Read the model definition and answer for the solid it produces. Units are mm, in the model's axes. A direction names the side the tool comes from. Round coordinates to 2 decimals unless told otherwise and drop trailing zeros. Loops run counter-clockwise (first coordinate to the right, second up) from the corner with the lowest first, then second, coordinate; pieces in that order, holes last. Notation, with made-up numbers: M 66,75 L 113,75 A34 ccw 113,114 Z; hole C 33,-29.5 d8. An arc over 180 degrees is marked long. Write each question's results on one line, items separated by ' | '.
```python
from build123d import *

# Parameters (mm, degrees)
SKETCH1_W                                         = 71.5
SKETCH1_H                                         = 30
SKETCH1_W_2                                       = 63.5
SKETCH1_H_2                                       = 22
BOSS_EXTRUDE1_DEPTH                               = 21
SKETCH2_W                                         = 71.5
SKETCH2_H                                         = 30
BOSS_EXTRUDE2_DEPTH                               = 3
SKETCH3_W                                         = 68.9
SKETCH3_H                                         = 27.4
SKETCH3_W_2                                       = 65.9
SKETCH3_H_2                                       = 24.4
CUT_EXTRUDE1_DEPTH                                = 1.5
SKETCH4_R                                         = 1.6
CUT_EXTRUDE2_DEPTH                                = 3
PILOT_HOLE_SIZE_PER_CROSS_FOR_HALF_CO_D           = 3.2
PILOT_HOLE_SIZE_PER_CROSS_FOR_HALF_CO_DEPTH       = 6.1
PILOT_HOLE_SIZE_PER_CROSS_FOR_HALF_CO_CSINK_D     = 6
PILOT_HOLE_SIZE_PER_CROSS_FOR_HALF_CO_CSINK_ANGLE = 90
PILOT_HOLE_SIZE_PER_CROSS_FOR_HALF_CO_TIP         = 0.96137699
FILLET1_R                                         = 1
FILLET2_R                                         = 1


with BuildPart() as part:
    # Sketch1 → Boss-Extrude1 (new body)
    with BuildSketch(Plane.XY):
        Rectangle(SKETCH1_W, SKETCH1_H)
        Rectangle(SKETCH1_W_2, SKETCH1_H_2, mode=Mode.SUBTRACT)
    extrude(amount=BOSS_EXTRUDE1_DEPTH)

    # Sketch2 → Boss-Extrude2 (add)
    with BuildSketch(Plane.XY.offset(21)):
        Polygon((42.25, 15), (42.25, -15), (42.25, -21.5), (-42.25, -21.5), (-42.25, -15), (-42.25, 15), (-42.25, 21.5), (42.25, 21.5), align=None)
        Rectangle(SKETCH2_W, SKETCH2_H, mode=Mode.SUBTRACT)
    extrude(amount=-BOSS_EXTRUDE2_DEPTH)

    # Sketch3 → Cut-Extrude1 (cut)
    with BuildSketch(Plane(origin=(0, 0, 0), x_dir=(-1, 0, 0), z_dir=(0, 0, -1))):
        Rectangle(SKETCH3_W, SKETCH3_H)
        Rectangle(SKETCH3_W_2, SKETCH3_H_2, mode=Mode.SUBTRACT)
    extrude(amount=-CUT_EXTRUDE1_DEPTH, mode=Mode.SUBTRACT)

    # Sketch4 → Cut-Extrude2 (cut)
    with BuildSketch(Plane(origin=(0, 0, 18), x_dir=(-1, 0, 0), z_dir=(0, 0, -1))):
        with Locations((-38.25, 16.5)):
            Circle(SKETCH4_R)
        with Locations((-38.25, -16.5)):
            Circle(SKETCH4_R)
        with Locations(Location((38.25, -16.5, 0), (0, 0, 180))):
            Circle(SKETCH4_R)
        with Locations(Location((38.25, 16.5, 0), (0, 0, 180))):
            Circle(SKETCH4_R)
        with Locations((0, -18)):
            Circle(SKETCH4_R)
        with Locations((0, 18)):
            Circle(SKETCH4_R)
    extrude(amount=-CUT_EXTRUDE2_DEPTH, mode=Mode.SUBTRACT)

    # Pilot hole size (% per cross) for half-countersunk wood screw, type 1
    with Locations(Plane.XY.offset(21)):
        with Locations((-38.25, 16.5), (-38.25, -16.5), (38.25, 16.5), (38.25, -16.5), (0, -18), (0, 18)):
            CounterSinkHole(PILOT_HOLE_SIZE_PER_CROSS_FOR_HALF_CO_D / 2, PILOT_HOLE_SIZE_PER_CROSS_FOR_HALF_CO_CSINK_D / 2, depth=PILOT_HOLE_SIZE_PER_CROSS_FOR_HALF_CO_DEPTH, counter_sink_angle=PILOT_HOLE_SIZE_PER_CROSS_FOR_HALF_CO_CSINK_ANGLE)
            with Locations((0, 0, -(PILOT_HOLE_SIZE_PER_CROSS_FOR_HALF_CO_DEPTH + PILOT_HOLE_SIZE_PER_CROSS_FOR_HALF_CO_TIP / 2))):  # 118° drill point
                Cone(0, PILOT_HOLE_SIZE_PER_CROSS_FOR_HALF_CO_D / 2, PILOT_HOLE_SIZE_PER_CROSS_FOR_HALF_CO_TIP, mode=Mode.SUBTRACT)

    # Fillet1
    fillet1_edges = [part.edges().sort_by_distance(p)[0] for p in [
        (-31.75, 11, 10.5),
        (-31.75, -11, 10.5),
        (31.75, -11, 10.5),
        (31.75, 11, 10.5),
        (34.45, 13.7, 0.75),
        (-34.45, 13.7, 0.75),
        (-34.45, -13.7, 0.75),
        (34.45, -13.7, 0.75),
        (32.95, -12.2, 0.75),
        (32.95, 12.2, 0.75),
        (-32.95, 12.2, 0.75),
        (-32.95, -12.2, 0.75),
    ]]
    fillet(fillet1_edges, radius=FILLET1_R)

    # Fillet2
    fillet2_edges = [part.edges().sort_by_distance(p)[0] for p in [
        (-35.75, -15, 9),
        (-35.75, 15, 9),
        (35.75, 15, 9),
        (35.75, -15, 9),
    ]]
    fillet(fillet2_edges, radius=FILLET2_R)


solid = part.part
```
1. Given P1, Ø1.6, axis at x = -2, z = 1, coming from the +Y side; P2, Ø3, axis at y = 11, z = 13.5, coming from the +X side; P3, Ø5, axis at x = -38.25, y = 16.5, coming from the +Z side, each flat-ended and moving along its own axis, determine where each tip first touches the part or whether it passes through.
Completed:
P1: stops at y = 15 | P2: stops at x = 35.75 | P3: stops at z = 20.5
2. Find the intervals of material crossed by L1, parallel to Y at x = -38.25, z = 19.2; L2, parallel to Y at x = 0, z = 19.15; L3, parallel to Y at x = 8.5, z = 2.5, in increasing order.
Completed:
L1: y = -21.5 to -18.1, -14.9 to 14.9, 18.1 to 21.5 | L2: y = -21.5 to -19.6, -16.4 to -11, 11 to 16.4, 19.6 to 21.5 | L3: y = -15 to -11, 11 to 15
3. Find section B-B, the plane x = 0. Count the separate pieces of the cut face and the enclosed holes in it, then the cut area to 3 significant figures.
Completed:
separate pieces: 4 | enclosed holes: 0 | area: 179 mm2
4. Find section C-C, the plane z = 12.5. Give the vertices of the cut face in (x, y).
Completed:
outline: M -35.75,-14 A1 ccw -34.75,-15 L 34.75,-15 A1 ccw 35.75,-14 L 35.75,14 A1 ccw 34.75,15 L -34.75,15 A1 ccw -35.75,14 Z; hole M -31.75,-10 A1 ccw -30.75,-11 L 30.75,-11 A1 ccw 31.75,-10 L 31.75,10 A1 ccw 30.75,11 L -30.75,11 A1 ccw -31.75,10 Z
5. Find section D-D, the plane x = 17. Give the vertices of the cut face in (y, z), then the cut area to 4 significant figures.
Completed:
outline: M -21.5,18 L -15,18 L -15,0 L -13.7,0 L -13.7,1.5 L -12.2,1.5 L -12.2,0 L -11,0 L -11,21 L -21.5,21 Z; M 11,0 L 12.2,0 L 12.2,1.5 L 13.7,1.5 L 13.7,0 L 15,0 L 15,18 L 21.5,18 L 21.5,21 L 11,21 Z | area: 202.5 mm2
6. Find section A-A, the plane y = -3.5. Give the vertices of the cut face in (x, z).
Completed:
outline: M -42.25,18 L -35.75,18 L -35.75,0 L -34.45,0 L -34.45,1.5 L -32.95,1.5 L -32.95,0 L -31.75,0 L -31.75,21 L -42.25,21 Z; M 31.75,0 L 32.95,0 L 32.95,1.5 L 34.45,1.5 L 34.45,0 L 35.75,0 L 35.75,18 L 42.25,18 L 42.25,21 L 31.75,21 Z
7. Which of the six approach directions +Z, -Z, +X, -X, +Y, -Y give full straight-line access (tool end or side, diameter ignored) to faces 1 (the face through (-35.75, 0, 9)), 2 (the face through (32.95, 0, 1)), 3 (the face through (0.208, 19.586, 18.789))?
Completed:
face 1: -Z, -X, +Y, -Y | face 2: -Z | face 3: +Z, -Z
8. Determine the mould class of faces 4 (the face through (-34.45, 0, 1)), 5 (the face through (1, -21.5, 20)), 6 (the face through (35.75, 0, 9)), 7 (the face through (0.208, -16.414, 18.789)) for opening direction Y: released by +Y, released by -Y, zero draft, split by the parting line, or undercut.
Completed:
face 4: undercut | face 5: released by -Y | face 6: zero draft | face 7: undercut
